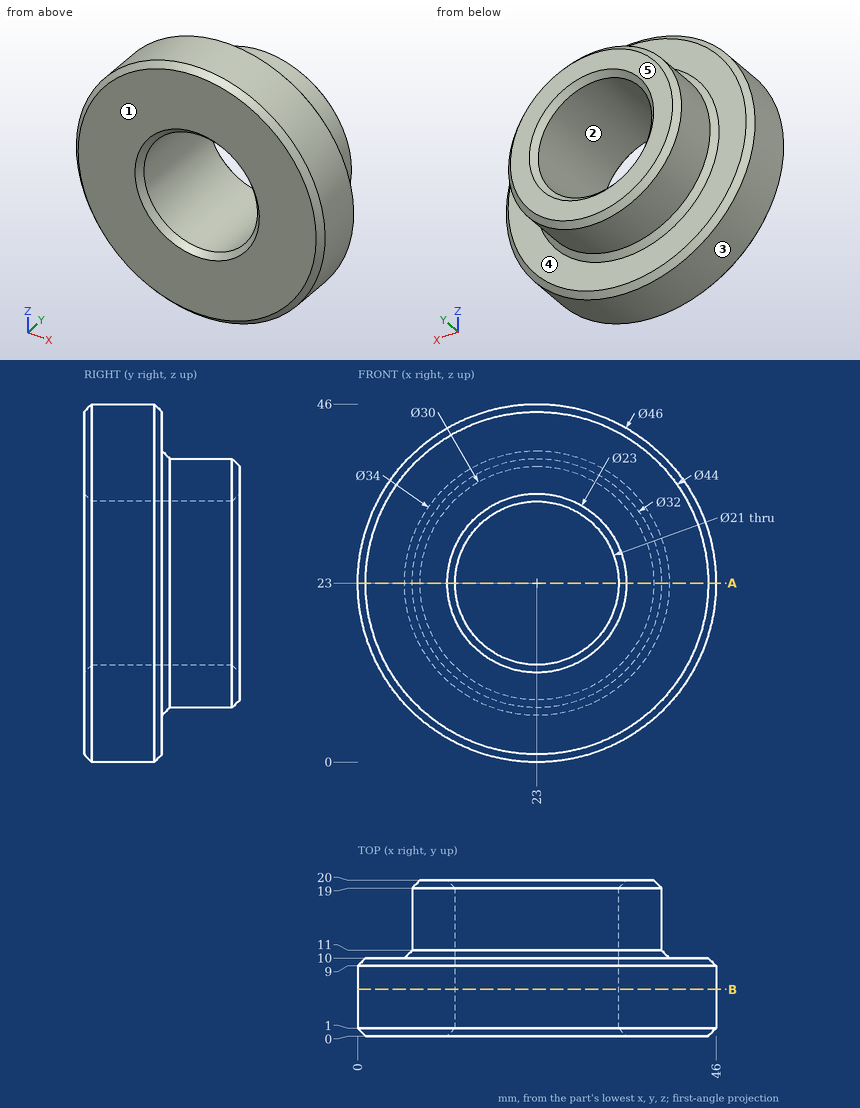
Verification items for this drawing (mm, ordinates from the low corner). A direction names the side the tool comes from. Coordinates: 2 decimals unless noted, no trailing zeros. Order: outer loops, then holes, each group sorted by start corner. A loop starts at its lowest first (then second) coordinate and runs counter-clockwise, first axis right, second up. Notation, with made-up numbers: (22, 71) -> (42, 71) arc R10 ccw to (42, 82) -> close; hole circle Ø6 at (-11, -4.5). An arc over 180 degrees is marked (long way). Answer as CSV lines item,"result". Start each with the question number.
1) Release check for a two-part mould opening along X. For the marked faces 1, 2 and 3 record: released by +X, released by -X, zero draft, split by the parting line, or undercut.
2) Gauge pin test, flat ends, axial feed: pin 1 Ø6 at (y, z) = (10.5, 7.5) entering from -X; pin 2 Ø5 at (y, z) = (14.5, 40) entering from +X; pin 3 Ø17 at (x, z) = (23, 23) entering from +Y; pin 4 Ø4 at (x, y) = (39, 17.5) entering from +Z. Record the tip position at first contact, or that the pin passes through.
3) Cross-section at B-B, the plane y = 6. Record the boundary of the cut face in (x, z), then the cut area to 3 significant figures.
4) Material ranges on L1, parallel to X at y = 6.75, z = 23; L2, parallel to Y at x = 41, z = 30; L3, parallel to Z at x = 31, y = 7.5, recorded low to high. Write a range as [from, to].
5) Cross-section at A-A, the plane z = 23. Record the boundary of the cut face in (x, y).
6) Set-up check for the marked faces 4 and 5: record each of +Z, -Z, +X, -X, +Y, -Y from which the full face is reachable in a straight line by a thin tool's end or side.
Conclusion:
1,face 1,"zero draft"
1,face 2,"undercut"
1,face 3,"split by the parting line"
2,pin 1,"stops at x = 3.96"
2,pin 2,"stops at x = 29.76"
2,pin 3,"passes through"
2,pin 4,"stops at z = 30.75"
3,outline,"circle Ø46 at (23, 23); hole circle Ø21 at (23, 23)"
3,area,"1,320 mm²"
4,L1,"x = [0, 12.5], [33.5, 46]"
4,L2,"y = [0, 10]"
4,L3,"z = [1.44, 16.2], [29.8, 44.56]"
5,outline,"(0, 1) -> (1, 0) -> (11.5, 0) -> (12.5, 1) -> (12.5, 19) -> (11.5, 20) -> (8, 20) -> (7, 19) -> (7, 11) -> (6, 10) -> (1, 10) -> (0, 9) -> close; (33.5, 1) -> (34.5, 0) -> (45, 0) -> (46, 1) -> (46, 9) -> (45, 10) -> (40, 10) -> (39, 11) -> (39, 19) -> (38, 20) -> (34.5, 20) -> (33.5, 19) -> close"
6,face 4,"+Y"
6,face 5,"+Z, -Z, +X, -X, +Y"
